Can you work these out from the model? Positions are in its coordinate system, mm. Face numbers are marked on the shaded views. Coordinates: 2 decimals unless noted, no trailing zeros. Answer in a Markdown table with one row per item.
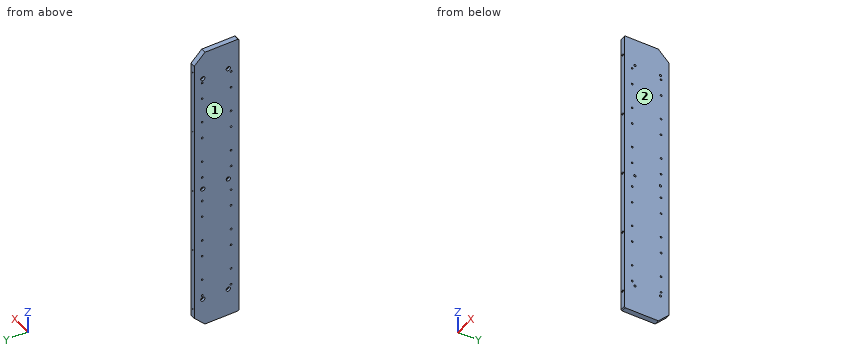
```python
from build123d import *

# Parameters (mm, degrees)
SKETCH_1_W                = 690
SKETCH_1_H                = 105
EXTRUDE_1_DEPTH           = 6
CHAMFER_1_SIZE            = 2
CHAMFER_2_SIZE            = 25
HOLE_WIZARD_M6_1_D        = 5
HOLE_WIZARD_M6_1_DEPTH    = 15
HOLE_WIZARD_M6_1_TIP      = 1.502151548
HOLE_WIZARD_1_D           = 5.5
HOLE_WIZARD_1_CBORE_D     = 10
HOLE_WIZARD_1_CBORE_DEPTH = 5.7
HOLE_WIZARD_M5_1_D        = 4.2
HOLE_WIZARD_M3_2_D        = 2.5
HOLE_WIZARD_M3_2_DEPTH    = 7.5
HOLE_WIZARD_M3_2_TIP      = 0.751075774


with BuildPart() as part:
    # 草图1 → 凸台-拉伸1 (new, symmetric)
    with BuildSketch(Plane(origin=(0, 0, 0), x_dir=(0, 0, -1), z_dir=(1, 0, 0))):
        Rectangle(SKETCH_1_W, SKETCH_1_H)
    extrude(amount=EXTRUDE_1_DEPTH, both=True)

    # 倒角1
    chamfer_1_edges = [part.edges().sort_by_distance(p)[0] for p in [
        (0, -52.5, -345),
        (0, -52.5, 345),
    ]]
    chamfer(chamfer_1_edges, length=CHAMFER_1_SIZE)

    # 倒角2
    chamfer_2_edges = [part.edges().sort_by_distance(p)[0] for p in [
        (0, 52.5, 345),
        (0, 52.5, -345),
    ]]
    chamfer(chamfer_2_edges, length=CHAMFER_2_SIZE)

    # M6 螺纹孔1
    with Locations(Plane(origin=(0, -52.5, 0), x_dir=(-1, 0, 0), z_dir=(0, -1, 0))):
        with Locations((0, -300), (0, -150), (0, 0), (0, 150), (0, 300)):
            Hole(HOLE_WIZARD_M6_1_D / 2, depth=HOLE_WIZARD_M6_1_DEPTH)
            with Locations((0, 0, -(HOLE_WIZARD_M6_1_DEPTH + HOLE_WIZARD_M6_1_TIP / 2))):  # 118° drill point
                Cone(0, HOLE_WIZARD_M6_1_D / 2, HOLE_WIZARD_M6_1_TIP, mode=Mode.SUBTRACT)

    # 打孔尺寸(%根据)内六角圆柱头螺钉的类型1 (through all)
    with Locations(Plane.ZY.offset(6)):
        with Locations((280, 32.5), (280, -27.5), (0, 32.5), (0, -27.5), (-280, 32.5), (-280, -27.5)):
            CounterBoreHole(HOLE_WIZARD_1_D / 2, HOLE_WIZARD_1_CBORE_D / 2, HOLE_WIZARD_1_CBORE_DEPTH)

    # M5 螺纹孔1 (through all)
    with Locations(Plane.ZY.offset(6)):
        with Locations((270, 34), (270, -34), (170, 34), (170, -34), (70, 34), (70, -34), (-30, 34), (-30, -34), (-130, 34), (-130, -34), (130, -34), (130, 34), (30, -34), (30, 34), (-70, -34), (-70, 34), (-170, -34), (-170, 34), (-270, -34), (-270, 34), (-230, 34), (-230, -34), (230, -34), (230, 34)):
            Hole(HOLE_WIZARD_M5_1_D / 2)

    # M3 螺纹孔2
    with Locations(Plane(origin=(0, 52.5, 0), x_dir=(1, 0, 0), z_dir=(0, 1, 0))):
        with Locations((0, -300), (0, -150), (0, 0), (0, 150), (0, 300)):
            Hole(HOLE_WIZARD_M3_2_D / 2, depth=HOLE_WIZARD_M3_2_DEPTH)
            with Locations((0, 0, -(HOLE_WIZARD_M3_2_DEPTH + HOLE_WIZARD_M3_2_TIP / 2))):  # 118° drill point
                Cone(0, HOLE_WIZARD_M3_2_D / 2, HOLE_WIZARD_M3_2_TIP, mode=Mode.SUBTRACT)


solid = part.part
```
(1) I need wall thicknesses on line 1 (Y direction, x = 2.75, z = -230); line 2 (Y direction, x = 3.25, z = 280); line 3 (X direction, y = 47, z = -300). Which ranges of each line are inside material? Lowest first, please. Write a range as [from, to].
Response values:
| item | result |
|---|---|
| line 1 | [-52.5, -36.1], [-31.9, 31.9], [36.1, 52.5] |
| line 2 | [-52.5, -30.25], [-24.75, 29.75], [35.25, 52.5] |
| line 3 | [-6, -1.25], [1.25, 6] |
(2) We'd pull the mould along X, two halves only. Please class the marked faces 1 and 2: +X half, -X half, draft (parallel to the pull), parting line (faces both ways), or undercut.
Response values:
| item | result |
|---|---|
| face 1 | -X half |
| face 2 | +X half |
(3) Will this pin go through, and if not, where does the flat tip stop? pin 1 Ø6.5 at (y, z) = (-27.5, -280) entering from -X.
Response values:
| item | result |
|---|---|
| pin 1 | x = -0.3 |
